from build123d import *

# Parameters (mm, degrees)
SKETCH1_R           = 60
BOSS_EXTRUDE1_DEPTH = 135
SKETCH2_R           = 30
BOSS_EXTRUDE2_DEPTH = 318
FILLET2_R           = 30
SKETCH3_R           = 26
BOSS_EXTRUDE3_DEPTH = 20


with BuildPart() as part:
    # Sketch1 → Boss-Extrude1 (new body)
    with BuildSketch(Plane.XY):
        with Locations((599.884196758, 0)):
            Circle(SKETCH1_R)
    extrude(amount=-BOSS_EXTRUDE1_DEPTH)

    # Sketch2 → Boss-Extrude2 (add)
    with BuildSketch(Plane(origin=(0, 0, -135), x_dir=(-1, 0, 0), z_dir=(0, 0, -1))):
        with Locations((-599.884196758, 0)):
            Circle(SKETCH2_R)
    extrude(amount=BOSS_EXTRUDE2_DEPTH)

    # Fillet2
    fillet2_edges = [part.edges().sort_by_distance(p)[0] for p in [
        (629.884196758, 0, -453),
    ]]
    fillet(fillet2_edges, radius=FILLET2_R)

    # Sketch3 → Boss-Extrude3 (add)
    with BuildSketch(Plane.XY.offset(-423)):
        with Locations((599.884196758, 0)):
            Circle(SKETCH3_R)
    extrude(amount=-BOSS_EXTRUDE3_DEPTH)


solid = part.part
Geometry: final body of the model. Coordinates: model frame, mm. A direction names the side the tool comes from. Coordinates: 2 decimals unless noted, no trailing zeros. Loops run counter-clockwise (first coordinate to the right, second up) from the corner with the lowest first, then second, coordinate; pieces in that order, holes last. Notation, with made-up numbers: (-20, 17.5) - (13, 17.5) arc R18 ccw to (13, 44.5) - close; hole circle Ø2 at (-38, 68). An arc over 180 degrees is marked (long way). Put each result on its own line as item: value. Start each with the question number.
Q1. Cut plane A-A, the plane y = 0. Return loops of the section in (x, z), and give its area (3 significant figures).
Q2. Cut plane C-C, the plane x = 594. Return loops of the section in (y, z), and give its area (3 significant figures).
Q3. Cut plane B-B, the plane z = -248. Return loops of the section in (x, y).
Q4. Pin query (flat end, axial travel): pin 1 Ø6 at (y, z) = (-4, -296) entering from -X; pin 2 Ø6 at (x, y) = (599, 33.5) entering from +Z; pin 3 Ø10 at (x, z) = (592, -208) entering from -Y; pin 4 Ø5 at (x, y) = (641, -41) entering from -Z. Return the tip coordinate at first contact, or that it passes through.
Q5. Cut plane D-D, the plane z = -45.5. Return loops of the section in (x, y).
Q6. Line query: line 1 (Z direction, x = 614, y = 44); line 2 (X direction, y = 1, z = -348.5); line 3 (Y direction, x = 615, z = -285). Output: solid intervals per line, ascending.
Q7. Set-up query: faces 1 (the flat face through (607.5, 21.3, -443)), 2 (the flat face through (599, 1, 0)). Return all of +Z, -Z, +X, -X, +Y, -Y with unobstructed straight access to the full face (end or side cutting, diameter ignored); none if empty.
Filled sheet:
1. outline: (539.88, -135) - (569.88, -135) - (569.88, -423) arc R30 ccw to (573.88, -437.97) - (573.88, -443) - (577.52, -443) arc R30 ccw to (622.24, -443) - (625.88, -443) - (625.88, -437.97) arc R30 ccw to (629.88, -423) - (629.88, -135) - (659.88, -135) - (659.88, 0) - (539.88, 0) - close
1. area: 34,900 mm²
2. outline: (-59.71, -135) - (-29.42, -135) - (-29.42, -423) arc R29.42 ccw to (-25.33, -437.97) - (-25.33, -443) - (-21.57, -443) arc R29.42 ccw to (21.57, -443) - (25.33, -443) - (25.33, -437.97) arc R29.42 ccw to (29.42, -423) - (29.42, -135) - (59.71, -135) - (59.71, 0) - (-59.71, 0) - close
2. area: 34,400 mm²
3. outline: circle Ø60 at (599.88, 0)
4. pin 1: x = 569.9
4. pin 2: z = 0
4. pin 3: y = -29.86
4. pin 4: z = -135
5. outline: circle Ø120 at (599.88, 0)
6. line 1: -135 to 0
6. line 2: 569.9 to 629.87
6. line 3: -25.91 to 25.91
7. face 1: -Z
7. face 2: +Z, +X, -X, +Y, -Y
